Can you work these out from the model? Positions are in its coordinate system, mm. A direction names the side the tool comes from. Give positions to 0.01 mm unless a question says otherwise; leave off trailing zeros. Order: outer loops, then holes, each group sorted by start corner. A loop starts at its lowest first (then second) coordinate and runs counter-clockwise, first axis right, second up. Notation, with made-up numbers: (16.25, 78) - (60.25, 78) arc R27 cw to (60.25, 111) - close; hole circle Ø6 at (77.25, 10.25). An arc over 180 degrees is marked (long way). Return JSON: item names as keys, results as strings.
```python
from build123d import *

# Parameters (mm, degrees)
BOSS_EXTRUDE1_DEPTH = 5
SKETCH2_R           = 5
BOSS_EXTRUDE2_DEPTH = 10
SKETCH3_W           = 9.261773254
SKETCH3_H           = 36.627775898
BOSS_EXTRUDE3_DEPTH = 4
SKETCH4_W           = 9.261773254
SKETCH4_H           = 8.313887949
BOSS_EXTRUDE4_DEPTH = 10
SKETCH5_R           = 7.423962758
BOSS_EXTRUDE5_DEPTH = 2
BOSS_EXTRUDE6_DEPTH = 3
SKETCH7_R           = 2.850666807
CUT_EXTRUDE1_DEPTH  = 0.1
CUT_EXTRUDE2_DEPTH  = 1


with BuildPart() as part:
    # Sketch1 → Boss-Extrude1 (new body)
    with BuildSketch(Plane(origin=(0, 0, 0), x_dir=(1, 0, 0), z_dir=(0, 1, 0))):
        Polygon((5.773502692, 10), (-5.773502692, 10), (-11.547005384, 0), (-5.773502692, -10), (5.773502692, -10), (11.547005384, 0), align=None)
    extrude(amount=BOSS_EXTRUDE1_DEPTH)

    # Sketch2 → Boss-Extrude2 (add)
    with BuildSketch(Plane.XZ):
        with Locations(Location((0.234789437, 0, 0), (0, 0, 270))):
            Circle(SKETCH2_R)
    extrude(amount=BOSS_EXTRUDE2_DEPTH)

    # Sketch3 → Boss-Extrude3 (add)
    with BuildSketch(Plane(origin=(0, 5, 0), x_dir=(1, 0, 0), z_dir=(0, 1, 0))):
        Rectangle(SKETCH3_W, SKETCH3_H)
    extrude(amount=BOSS_EXTRUDE3_DEPTH)

    # Sketch4 → Boss-Extrude4 (add)
    with BuildSketch(Plane(origin=(0, 9, 0), x_dir=(1, 0, 0), z_dir=(0, 1, 0))):
        with Locations((0, 14.156943975)):
            Rectangle(SKETCH4_W, SKETCH4_H)
        with Locations((0, -14.156943975)):
            Rectangle(SKETCH4_W, SKETCH4_H)
    extrude(amount=BOSS_EXTRUDE4_DEPTH)

    # Sketch5 → Boss-Extrude5 (add)
    with BuildSketch(Plane(origin=(0, 9, 0), x_dir=(1, 0, 0), z_dir=(0, 1, 0))):
        with Locations(Location((0, 0, 0), (0, 0, 51.407625877))):
            Circle(SKETCH5_R)
    extrude(amount=BOSS_EXTRUDE5_DEPTH)

    # Sketch6 → Boss-Extrude6 (add)
    with BuildSketch(Plane(origin=(0, 11, 0), x_dir=(1, 0, 0), z_dir=(0, 1, 0))):
        Polygon((0, 4.871086868), (-4.218484972, 2.435543434), (-4.218484972, -2.435543434), (0, -4.871086868), (4.218484972, -2.435543434), (4.218484972, 2.435543434), align=None)
    extrude(amount=BOSS_EXTRUDE6_DEPTH)

    # Sketch7 → Cut-Extrude1 (cut)
    with BuildSketch(Plane(origin=(0, 19, 0), x_dir=(1, 0, 0), z_dir=(0, 1, 0))):
        with Locations(Location((0, 14.250511049, 0), (0, 0, 270))):
            Circle(SKETCH7_R)
        with Locations(Location((0, -14.372767949, 0), (0, 0, 270))):
            Circle(SKETCH7_R)
    extrude(amount=-CUT_EXTRUDE1_DEPTH, mode=Mode.SUBTRACT)

    # Sketch8 → Cut-Extrude2 (cut)
    with BuildSketch(Plane(origin=(0, 18.9, 0), x_dir=(1, 0, 0), z_dir=(0, 1, 0))):
        Polygon((-1.343066927, 11.719300444), (0.804329856, 17.000767289), (1.330666503, 16.786763555), (-0.81673028, 11.505296711), align=None)
        Polygon((-1.076876675, -17.027451515), (0.531783037, -11.557769723), (1.076876675, -11.718084383), (-0.531783037, -17.187766175), align=None)
    extrude(amount=-CUT_EXTRUDE2_DEPTH, mode=Mode.SUBTRACT)


solid = part.part
```
1. On a 3-axis mill with a long thin cutter (end or side, diameter ignored), from which of +Z, -Z, +X, -X, +Y, -Y can I reach the whole of each face in a straight line? I mean faces 4 (the face through (-4.646, -4.93, 1.084)), 5 (the face through (-2.08, 12.48, -3.67)), 6 (the face through (1, 18.9, 15)), 7 (the face through (0, 14, -10)), 8 (the face through (0, 5, 14)). Say none if no direction works.
Checks:
{"face 4": "-Y", "face 5": "-X, +Y", "face 6": "+Y", "face 7": "+X, -X, +Y", "face 8": "+Z, +X, -X, -Y"}
2. Thinking about a two-plate mould opening in Y: for faces 1 (the face through (-7, 5, 0)), 2 (the face through (0, 14, 0)), 3 (the face through (0, 14, 10)), which applies, +Y half, -Y half, draft (parallel to the pull), parting line (faces both ways), or undercut?
Checks:
{"face 1": "undercut", "face 2": "+Y half", "face 3": "draft"}
3. For pin 1 Ø5 at (x, z) = (0, 14.37) entering from +Y; pin 2 Ø7 at (y, z) = (13.5, -2.5) entering from +X; pin 3 Ø3.5 at (x, z) = (-7, -3) entering from +Y; pin 4 Ø4 at (x, y) = (1, 3.5) entering from +Z, each with a flat end and sliding along its axis, tell me the tip position at first contact or that it passes through.
Checks:
{"pin 1": "y = 18.9", "pin 2": "x = 7.42", "pin 3": "y = 11", "pin 4": "z = 18.31"}
4. Suppose I cut it at C-C (x = -5.25). List the corners of the cut face in (y, z) for me.
Checks:
{"outline": "(0, -10) - (5, -10) - (5, 10) - (0, 10) - close; (9, -5.25) - (11, -5.25) - (11, 5.25) - (9, 5.25) - close"}
5. Suppose I cut it at B-B (y = 10.25). List the corners of the cut face in (x, z) for me.
Checks:
{"outline": "circle Ø14.85 at (0, 0); (-4.63, -18.31) - (4.63, -18.31) - (4.63, -10) - (-4.63, -10) - close; (-4.63, 10) - (4.63, 10) - (4.63, 18.31) - (-4.63, 18.31) - close"}
6. Suppose I cut it at D-D (z = -9.5). List the corners of the cut face in (x, y) for me.
Checks:
{"outline": "(-6.06, 0) - (6.06, 0) - (6.06, 5) - (4.63, 5) - (4.63, 9) - (-4.63, 9) - (-4.63, 5) - (-6.06, 5) - close"}
7. Suppose I cut it at A-A (y = 16). List the corners of the cut face in (x, z) for me, plus the area to 3 significant figures.
Checks:
{"outline": "(-4.63, -18.31) - (4.63, -18.31) - (4.63, -10) - (-4.63, -10) - close; (-4.63, 10) - (4.63, 10) - (4.63, 18.31) - (-4.63, 18.31) - close", "area": "154 mm^2"}
8. If I drill on L1, parallel to Z at x = 0, y = 18.95; L2, parallel to Y at x = 5, z = 2.5; L3, parallel to Z at x = -4.5, y = 14.75, over which ranges is the centre line in solid material (lowest first)? Write a range as [from, to].
Checks:
{"L1": "[-18.31, -17.1], [-11.4, -10], [10, 11.52], [17.22, 18.31]", "L2": "[0, 5], [9, 11]", "L3": "[-18.31, -10], [10, 18.31]"}
